from build123d import *


with BuildPart() as part:
    # Sketch1 → Revolve1 (revolve)
    with BuildSketch(Plane(origin=(0, 0, 0), x_dir=(0, 0, -1), z_dir=(1, 0, 0)), mode=Mode.PRIVATE) as revolve1_sk:
        with BuildLine():
            Line((-237.998, 63.5), (-153.9875, 63.5))
            ThreePointArc((-153.9875, 63.5), (-152.864967985, 63.964967985), (-152.4, 65.0875))
            Line((-152.4, 65.0875), (-152.4, 76.073))
            Line((-152.4, 76.073), (-149.098, 79.375))
            Line((-149.098, 79.375), (-120.65, 79.375))
            Line((-120.65, 79.375), (-120.65, 72.2376))
            ThreePointArc((-120.65, 72.2376), (-120.185032015, 71.115067985), (-119.0625, 70.6501))
            Line((-119.0625, 70.6501), (-104.40462327, 70.6501))
            Line((-104.40462327, 70.6501), (-101.6, 72.26935))
            Line((-101.6, 72.26935), (150.114, 72.26935))
            Line((150.114, 72.26935), (152.4, 70.949527285))
            Line((152.4, 70.949527285), (152.4, 63.5))
            Line((152.4, 63.5), (237.998, 63.5))
            Line((237.998, 63.5), (241.3, 60.198))
            Line((241.3, 60.198), (241.3, 0))
            Line((241.3, 0), (-241.3, 0))
            Line((-241.3, 0), (-241.3, 60.198))
            Line((-241.3, 60.198), (-237.998, 63.5))
        make_face()
    revolve(revolve1_sk.sketch.rotate(Axis((0, 0, 264.578884175), (0, 0, -1)), 90), axis=Axis((0, 0, 264.578884175), (0, 0, -1)))


solid = part.part
Could you check a few things on this model? Use its own coordinates, in mm. A direction names the side the tool comes from. Coordinates: 2 decimals unless noted, no trailing zeros. Order: outer loops, then holes, each group sorted by start corner. A loop starts at its lowest first (then second) coordinate and runs counter-clockwise, first axis right, second up.
Q1. Please list where these lines run through material, in increasing order: L1, parallel to X at y = 15.5, z = -79; L2, parallel to Z at x = -60.5, y = 36.
Q2. Which directions (+Z, -Z, +X, -X, +Y, -Y) give clear straight access to the entire face, cutting with the end or side of a thin tool? Please do faces 4 (the flat face through (-53, 36, -152.4)), 5 (the flat face through (-1, -1, -241.3)), 6 (the flat face through (-56, -34, 152.4)), 7 (the conical face through (-15.34, 69.07, 104.23)).
Q3. Will these pins go through, and if not, where does the flat tip stop? pin 1 (8 mm diameter, centred on x = -31.5, z = -48.5, fed in from +Y); pin 2 (1 mm diameter, centred on y = -31.5, z = 41.5, fed in from -X); pin 3 (12 mm diameter, centred on y = 26, z = 109.5, fed in from +X).
Q4. Thinking about a two-plate mould opening in Z: for faces 1 (the conical face through (-16.54, 74.47, 152.19)), 2 (the cylindrical face through (-13.77, 61.99, 195.4)), 3 (the cylindrical face through (32.6, 62.68, 111.63)), which applies, released by +Z, released by -Z, zero draft, split by the parting line, or undercut?
Q5. Suppose I cut it at D-D on z = 209. Please give me the cut outline in (x, y).
Q6. Suppose I cut it at C-C on z = -112. Please give me the cut outline in (x, y), and give its area (3 significant figures).
Answer:
1. L1: x = -70.59 to 70.59
1. L2: z = -152.4 to 152.4
2. face 4: -Z
2. face 5: -Z, +X, -X, +Y, -Y
2. face 6: +Z
2. face 7: none
3. pin 1: stops at y = 66.83
3. pin 2: stops at x = -65.28
3. pin 3: stops at x = 67.76
4. face 1: released by +Z
4. face 2: zero draft
4. face 3: undercut
5. outline: circle Ø127 at (0, 0)
6. outline: circle Ø144.54 at (0, 0)
6. area: 16,400 mm2
